Verification items for the finished model (mm, model axes). A direction names the side the tool comes from. Coordinates: 2 decimals unless noted, no trailing zeros. Order: outer loops, then holes, each group sorted by start corner. A loop starts at its lowest first (then second) coordinate and runs counter-clockwise, first axis right, second up. Notation, with made-up numbers: M 8,13 L 16,13 A8 cw 16,23 Z; hole C -15.75,-8.75 d5. An arc over 180 degrees is marked long. Return JSON: item names as keys, results as strings. Group by question number.
1. Section check B-B, the plane x = 13.5. Record the cut outline in (y, z).
2. Set-up check for faces 1 (the flat face through (5, 0, -12)), 2 (the flat face through (9.2, -6, 11)), 3 (the flat face through (9.2, 6, -11)), 4 (the conical face through (0.26, 12.45, -0.03)), 5 (the flat face through (10, -8, 5)): record each of +Z, -Z, +X, -X, +Y, -Y from which the full face is reachable in a straight line by a thin tool's end or side.
3. Gauge pin test, flat ends, axial feed: pin 1 (6 mm diameter, centred on x = 30, z = -9.5, fed in from -Y); pin 2 (12 mm diameter, centred on y = -6, z = 4.5, fed in from +X); pin 3 (1.5 mm diameter, centred on y = 12, z = -1, fed in from +X); pin 4 (8 mm diameter, centred on x = 14.5, z = -9.5, fed in from -Y). Record the tip position at first contact, or that the pin passes through.
4. Material ranges on line 1 along X through (y, z) = (9.25, -5.75); line 2 along Z through (x, y) = (33, -3); line 3 along X through (y, z) = (-12.5, 1.5), recorded low to high.
5. Section check A-A, the plane x = 8.5. Record the cut outline in (y, z).
```python
from build123d import *

# Parameters (mm, degrees)
BASE_EXTRUDE_DEPTH = 10
SKETCH4_W          = 0.8
SKETCH4_H          = 11.856406461
CHAMFER_2_SIZE     = 1.6
FILLET_2_R         = 0.6


with BuildPart() as part:
    # Sketch1 → Base-Extrude (new body)
    with BuildSketch(Plane(origin=(0, 0, 0), x_dir=(0, 0, -1), z_dir=(1, 0, 0))):
        Polygon((12, 6.92820323), (12, -6.92820323), (0, -13.856406461), (-12, -6.92820323), (-12, 6.92820323), (0, 13.856406461), align=None)
    extrude(amount=BASE_EXTRUDE_DEPTH)

    # Sketch2 → Boss-Revolve1 (revolve)
    with BuildSketch(Plane.XY, mode=Mode.PRIVATE) as boss_revolve1_sk:
        Polygon((0, 0), (35.4, 0), (35.4, 6.268), (35.4, 8), (27.8072, 8), (0, 8), align=None)
    revolve(boss_revolve1_sk.sketch.rotate(Axis((0, 0, 0), (1, 0, 0)), 90), axis=Axis((0, 0, 0), (1, 0, 0)))

    # Sketch3 → Cut-Revolve1 (revolve, cut)
    with BuildSketch(Plane.XY):
        Polygon((0, 12), (3.958548116, 18.856406461), (3.958548116, 23.856406461), (-10, 23.856406461), (-10, 12), align=None)
    revolve(axis=Axis((0, 0, 0), (1, 0, 0)), mode=Mode.SUBTRACT)

    # Sketch5 → Cut-Revolve2 (revolve, cut)
    with BuildSketch(Plane.XY):
        Polygon((10, 12), (6.041451884, 18.856406461), (6.041451884, 23.856406461), (16.041451884, 23.856406461), (16.041451884, 12), align=None)
    revolve(axis=Axis((0, 0, 0), (1, 0, 0)), mode=Mode.SUBTRACT)

    # Sketch4 → Cut-Revolve3 (revolve, cut)
    with BuildSketch(Plane.XY, mode=Mode.PRIVATE) as cut_revolve3_sk:
        with Locations((9.6, 17.928203231)):
            Rectangle(SKETCH4_W, SKETCH4_H)
    revolve(cut_revolve3_sk.sketch.rotate(Axis((0, 0, 0), (1, 0, 0)), 270), axis=Axis((0, 0, 0), (1, 0, 0)), mode=Mode.SUBTRACT)

    # Chamfer 2
    chamfer_2_edges = [part.edges().sort_by_distance(p)[0] for p in [
        (35.4, 0, -8),
    ]]
    chamfer(chamfer_2_edges, length=CHAMFER_2_SIZE)

    # Fillet 2
    fillet_2_edges = [part.edges().sort_by_distance(p)[0] for p in [
        (10, 0, -8),
    ]]
    fillet(fillet_2_edges, radius=FILLET_2_R)


solid = part.part
```
Answers follow:
{
 "1": {"outline": "C 0,0 d16"},
 "2": {"face 1": "-Z, +X, -X, +Y, -Y", "face 2": "+Z, +X, -Y", "face 3": "-Z, +X, +Y", "face 4": "-X, +Y", "face 5": "+X"},
 "3": {"pin 1": "y = -4.66", "pin 2": "x = 35.4", "pin 3": "x = 10", "pin 4": "y = -5.81"},
 "4": {"line 1": "0 to 10", "line 2": "-7.42 to 7.42", "line 3": "0.34 to 9.2"},
 "5": {"outline": "M -13.86,0 L -6.93,-12 L 6.93,-12 L 13.86,0 L 6.93,12 L -6.93,12 Z"}
}
